Here's how the part is built. I have some questions about the finished solid (model axes, mm). A direction names the side the tool comes from. Coordinates: 2 decimals unless noted, no trailing zeros. Order: outer loops, then holes, each group sorted by start corner. A loop starts at its lowest first (then second) coordinate and runs counter-clockwise, first axis right, second up. Notation, with made-up numbers: (70, -23) - (94, -23) arc R21 cw to (94, 0) - close; hole circle Ø7 at (71.5, -22.5). An arc over 180 degrees is marked (long way). Answer as CSV lines item,"result". Start each with the question number.
Q1. For faces 1 (the face through (-239.37, -48.97, 7.04)), 2 (the face through (-240.89, -46.34, 1.97)), 3 (the face through (-99, 2, 10)), which set-ups out of +Z, -Z, +X, -X, +Y, -Y let a thin tool reach every point of the face, with its end or its side?
Q2. Suppose I cut it at A-A (x = 57). Please give me the cut outline in (y, z).
Q3. Suppose I cut it at B-B (z = 6.75). Please give me the cut outline in (x, y).
Q4. Suppose I cut it at D-D (y = -110). Please give me the cut outline in (x, z), then the cut area to 3 significant figures.
Q5. Thinking about a two-plate mould opening in X: for faces 4 (the face through (-241.48, 12.68, 1.97)), 5 (the face through (62, 19.52, 4.93)), 6 (the face through (-100, 2, 0)), 7 (the face through (-57.61, -109.15, 7.04)), which applies, released by +X, released by -X, zero draft, split by the parting line, or undercut?
Q6. For pin 1 Ø5 at (x, z) = (-63, 2) entering from -Y, with a flat end and sliding along its axis, tell me the tip position at first contact or that it passes through.
Q7. Suppose I cut it at C-C (x = -224.5). Please give me the cut outline in (y, z), then the cut area to 3 significant figures.
Q8. I need wall thicknesses on line 1 (X direction, y = -42, z = 8.25); line 2 (Y direction, x = 133, z = 4.25); line 3 (X direction, y = -7.5, z = 1). Which ranges of each line are inside material? Lowest first, please.
from build123d import *

# Parameters (mm, degrees)
SKETCH1_R           = 65
BOSS_EXTRUDE1_DEPTH = 10
CHAMFER1_SIZE       = 6


with BuildPart() as part:
    # Sketch1 → Boss-Extrude1 (new body)
    with BuildSketch(Plane.XY):
        with BuildLine():
            Line((-262.3, 130.8), (-262.3, 24.7))
            Line((-262.3, 24.7), (-220.073481324, 0.320508076))
            ThreePointArc((-220.073481324, 0.320508076), (-210.073481324, -17), (-220.073481324, -34.320508076))
            Line((-220.073481324, -34.320508076), (-262.3, -58.7))
            Line((-262.3, -58.7), (-262.3, -130.8))
            Line((-262.3, -130.8), (153.441030377, -93.022753927))
            ThreePointArc((153.441030377, -93.022753927), (160.218033303, -89.465947057), (162.495055771, -82.158840075))
            Line((162.495055771, -82.158840075), (160.91140277, -64.73063662))
            ThreePointArc((160.91140277, -64.73063662), (90, 0), (160.91140277, 64.73063662))
            Line((160.91140277, 64.73063662), (162.495055771, 82.158840075))
            ThreePointArc((162.495055771, 82.158840075), (160.218033303, 89.465947057), (153.441030377, 93.022753927))
            Line((153.441030377, 93.022753927), (-262.3, 130.8))
        make_face()
        Circle(SKETCH1_R, mode=Mode.SUBTRACT)
    extrude(amount=BOSS_EXTRUDE1_DEPTH)

    # Chamfer1
    chamfer1_edges = [part.edges().sort_by_distance(p)[0] for p in [
        (160.218033303, -89.465947057, 10),
        (161.703229271, -73.444738348, 10),
        (90, 0, 10),
        (161.703229271, 73.444738348, 10),
        (160.218033303, 89.465947057, 10),
        (-54.429484811, 111.911376963, 10),
        (-262.3, 77.75, 10),
        (-241.186740662, 12.510254038, 10),
        (-210.073481324, -17, 10),
        (-241.186740662, -46.510254038, 10),
        (-262.3, -94.75, 10),
        (-54.429484811, -111.911376963, 10),
    ]]
    chamfer(chamfer1_edges, length=CHAMFER1_SIZE)


solid = part.part
Here are the results:
1,face 1,"+Z, -X"
1,face 2,"+Z, -Z, -X"
1,face 3,"+Z, +X, -X, +Y, -Y"
2,outline,"(-101.79, 0) - (-31.24, 0) - (-31.24, 10) - (-95.76, 10) - (-101.79, 4) - close; (31.24, 0) - (101.79, 0) - (101.79, 4) - (95.76, 10) - (31.24, 10) - close"
3,outline,"(-259.55, -127.79) - (153.19, -90.28) arc R7.25 ccw to (159.76, -82.41) - (158.42, -67.66) arc R67.75 cw (long way) to (158.42, 67.66) - (159.76, 82.41) arc R7.25 ccw to (153.19, 90.28) - (-259.55, 127.79) - (-259.55, 26.29) - (-218.7, 2.7) arc R22.75 cw to (-218.7, -36.7) - (-259.55, -60.29) - close; hole circle Ø130 at (0, 0)"
4,outline,"(-262.3, 0) - (-33.39, 0) - (-33.39, 4) - (-99.7, 10) - (-256.3, 10) - (-262.3, 4) - close"
4,area,"2,070 mm²"
5,face 4,"released by -X"
5,face 5,"undercut"
5,face 6,"zero draft"
5,face 7,"released by +X"
6,pin 1,"stops at y = -112.92"
7,outline,"(-127.37, 0) - (-36.88, 0) - (-36.88, 4) - (-43.8, 10) - (-121.34, 10) - (-127.37, 4) - close; (2.88, 0) - (127.37, 0) - (127.37, 4) - (121.34, 10) - (9.8, 10) - (2.88, 4) - close"
7,area,"2,070 mm²"
8,line 1,"x = -224.87 to -49.61, 49.61 to 99.94"
8,line 2,"y = -94.63 to -61.43, 61.43 to 94.63"
8,line 3,"x = -212.47 to -64.57, 64.57 to 90.43"
